from build123d import *

# Parameters (mm, degrees)
CENTRE_BLOCK_PROFILE_W = 70
CENTRE_BLOCK_PROFILE_H = 40
CENTRE_BLOCK_DEPTH     = 30
END_LOOPS_DEPTH        = 25
CROSS_HOLE_PROFILE_R   = 7.5
CROSS_HOLE_15_DEPTH    = 95


with BuildPart() as part:
    # Centre Block Profile → Centre Block (new body)
    with BuildSketch(Plane.XY):
        Rectangle(CENTRE_BLOCK_PROFILE_W, CENTRE_BLOCK_PROFILE_H)
        with BuildLine():
            Line((20, -10), (-20, -10))
            ThreePointArc((-20, -10), (-30, 0), (-20, 10))
            Line((-20, 10), (20, 10))
            ThreePointArc((20, 10), (30, 0), (20, -10))
        make_face(mode=Mode.SUBTRACT)
    extrude(amount=CENTRE_BLOCK_DEPTH)

    # End Loops Profile → End Loops (add, symmetric)
    # profile 1 of 2: a face of its own
    with BuildSketch(Plane.XY.offset(15)):
        with BuildLine():
            Line((65, 30), (65, -30))
            ThreePointArc((65, -30), (50, -45), (35, -30))
            Line((35, -30), (35, 30))
            ThreePointArc((35, 30), (50, 45), (65, 30))
        make_face()
        with BuildLine():
            Line((60, 30), (60, -30))
            ThreePointArc((60, -30), (50, -40), (40, -30))
            Line((40, -30), (40, 30))
            ThreePointArc((40, 30), (50, 40), (60, 30))
        make_face(mode=Mode.SUBTRACT)
    # profile 2 of 2: a face of its own
    with BuildSketch(Plane.XY.offset(15)):
        with BuildLine():
            Line((-65, 30), (-65, -30))
            ThreePointArc((-65, -30), (-50, -45), (-35, -30))
            Line((-35, -30), (-35, 30))
            ThreePointArc((-35, 30), (-50, 45), (-65, 30))
        make_face()
        with BuildLine():
            Line((-40, 30), (-40, -30))
            ThreePointArc((-40, -30), (-50, -40), (-60, -30))
            Line((-60, -30), (-60, 30))
            ThreePointArc((-60, 30), (-50, 40), (-40, 30))
        make_face(mode=Mode.SUBTRACT)
    extrude(amount=END_LOOPS_DEPTH, both=True)

    # Cross Hole Profile → Cross Hole Ø15 (cut, symmetric)
    with BuildSketch(Plane(origin=(0, 0, 0), x_dir=(0, 0, -1), z_dir=(1, 0, 0))):
        with Locations(Location((-15, 0, 0), (0, 0, 270))):
            Circle(CROSS_HOLE_PROFILE_R)
    extrude(amount=CROSS_HOLE_15_DEPTH, both=True, mode=Mode.SUBTRACT)


solid = part.part
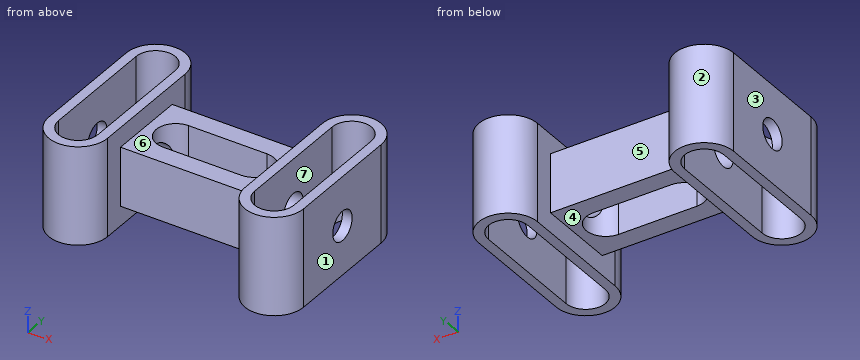
Design review of the part built by this model. Coordinates are the model's own, in mm. Face numbers are marked on the shaded views. A direction names the side the tool comes from. Give positions to 0.01 mm unless a question says otherwise; leave off trailing zeros. Write each loop counter-clockwise with the first axis right and the second up, starting at its lowest first coordinate (ties: lowest second). Pieces come first, ordered by that corner, then holes. Notation, with made-up numbers: M -20.5,31.25 L 1.5,31.25 A22 ccw 1.5,51.25 Z; hole C 1.25,61 d7. An arc over 180 degrees is marked long. Return JSON: item names as keys, results as strings. Group by question number.
Item 1: Tool access review of the marked faces 4, 5, 6 and 7: name each direction out of +Z, -Z, +X, -X, +Y, -Y from which nothing blocks a thin tool from reaching the whole face with its end or side.
Item 2: Wall thickness on line 1 along X through (y, z) = (19, 10); line 2 along X through (y, z) = (-24.5, -0.5); line 3 along Z through (x, y) = (-32, 0): over which ranges is each line inside the solid? List them lowest first.
Item 3: Take a section at B-B (y = 15). Give the boundary of the cut face in (x, z).
Item 4: Take a section at C-C (x = 15.5). Give the boundary of the cut face in (y, z).
Item 5: Take a section at D-D (x = -50). Give the boundary of the cut face in (y, z), plus the area to 3 significant figures.
Item 6: The part is to be moulded in two halves that separate along X. For the marked faces 1, 2 and 3, say which applies: pulls with the +X half, pulls with the -X half, needs draft (parallel to the pull), parting line crosses it, or undercut.
Item 7: Clearance check with flat-ended pins moving along their axes: pin 1 Ø10 at (x, y) = (3, 22.5) entering from -Z; pin 2 Ø5 at (x, z) = (4.5, 8.5) entering from -Y; pin 3 Ø12 at (x, z) = (-24, 8) entering from +Y. State where each tip first meets the part, or that it passes through.
Item 8: Take a section at A-A (z = 36). Give the boundary of the cut face in (x, y).
Return value:
{
 "1": {"face 4": "-Z, +Y, -Y", "face 5": "+Z, -Z, +Y", "face 6": "+Z, +Y, -Y", "face 7": "+Z, -Z"},
 "2": {"line 1": "x = -65 to -60, -40 to 40, 60 to 65", "line 2": "x = -65 to -60, -40 to -35, 35 to 40, 60 to 65", "line 3": "z = 0 to 7.5, 22.5 to 30"},
 "3": {"outline": "M -65,-10 L -60,-10 L -60,40 L -65,40 Z; M -40,-10 L -35,-10 L -35,0 L 35,0 L 35,-10 L 40,-10 L 40,40 L 35,40 L 35,30 L -35,30 L -35,40 L -40,40 Z; M 60,-10 L 65,-10 L 65,40 L 60,40 Z"},
 "4": {"outline": "M -20,0 L -10,0 L -10,30 L -20,30 Z; M 10,0 L 20,0 L 20,30 L 10,30 Z"},
 "5": {"outline": "M -45,-10 L -40,-10 L -40,40 L -45,40 Z; M 40,-10 L 45,-10 L 45,40 L 40,40 Z", "area": "500 mm2"},
 "6": {"face 1": "pulls with the +X half", "face 2": "undercut", "face 3": "pulls with the -X half"},
 "7": {"pin 1": "stops at z = 0", "pin 2": "stops at y = -20", "pin 3": "stops at y = 20"},
 "8": {"outline": "M -65,-30 A15 ccw -35,-30 L -35,30 A15 ccw -65,30 Z; M 35,-30 A15 ccw 65,-30 L 65,30 A15 ccw 35,30 Z; hole M -60,-30 A10 ccw -40,-30 L -40,30 A10 ccw -60,30 Z; hole M 40,-30 A10 ccw 60,-30 L 60,30 A10 ccw 40,30 Z"}
}
